CAD build for the part. Positions are in the model's coordinates, mm. A direction names the side the tool comes from. Give positions to 0.01 mm unless a question says otherwise; leave off trailing zeros. Loops run counter-clockwise (first coordinate to the right, second up) from the corner with the lowest first, then second, coordinate; pieces in that order, holes last. Notation, with made-up numbers: (-12, -16.75) - (2, -16.75) arc R14 cw to (2, -1.75) - close; hole circle Ø4 at (21, 28.5). An arc over 180 degrees is marked (long way). Return JSON: item names as keys, results as strings.
from build123d import *

# Parameters (mm, degrees)
SKETCH7_R              = 11
BOSS_EXTRUDE1_DEPTH    = 2.5
SKETCH8_R              = 8.75
SKETCH8_R_2            = 7.6
BOSS_EXTRUDE2_DEPTH    = 1
M14X1_5_TAPPED_HOLE1_D = 12.5
SKETCH13_OUTSIDE_W     = 30.338
SKETCH13_OUTSIDE_H     = 30.338
SKETCH13_OUTSIDE_W_2   = 20
SKETCH13_OUTSIDE_H_2   = 20
CUT_EXTRUDE1_DEPTH     = 17.673332001
M3_TAPPED_HOLE3_REACH  = 24.633
M3_TAPPED_HOLE3_BORE_R = 1.25


with BuildPart() as part:
    # Sketch7 → Boss-Extrude1 (new, symmetric)
    with BuildSketch(Plane.XY):
        Circle(SKETCH7_R)
    extrude(amount=BOSS_EXTRUDE1_DEPTH, both=True)

    # Sketch8 → Boss-Extrude2 (add)
    with BuildSketch(Plane.XY.offset(2.5)):
        Circle(SKETCH8_R)
        Circle(SKETCH8_R_2, mode=Mode.SUBTRACT)
    extrude(amount=BOSS_EXTRUDE2_DEPTH)

    # M14x1.5 Tapped Hole1 (through all)
    with Locations(Plane(origin=(0, 0, -2.5), x_dir=(-1, 0, 0), z_dir=(0, 0, -1))):
        with Locations((0, 0)):
            Hole(M14X1_5_TAPPED_HOLE1_D / 2)

    # Sketch13 outside → Cut-Extrude1 (cut, through all)
    with BuildSketch(Plane(origin=(0, 0, -2.5), x_dir=(-1, 0, 0), z_dir=(0, 0, -1))):
        Rectangle(SKETCH13_OUTSIDE_W, SKETCH13_OUTSIDE_H)
        Rectangle(SKETCH13_OUTSIDE_W_2, SKETCH13_OUTSIDE_H_2, mode=Mode.SUBTRACT)
    extrude(amount=-CUT_EXTRUDE1_DEPTH, mode=Mode.SUBTRACT)

    # M3 Tapped Hole3 bore → M3 Tapped Hole3 (cut, up to next)
    with BuildSketch(Plane(origin=(0, 10, 0), x_dir=(1, 0, 0), z_dir=(0, 1, 0)), mode=Mode.PRIVATE) as m3_tapped_hole3_sk1:
        Circle(M3_TAPPED_HOLE3_BORE_R)
    m3_tapped_hole3_tool1 = extrude(m3_tapped_hole3_sk1.sketch, amount=-M3_TAPPED_HOLE3_REACH, mode=Mode.PRIVATE) & part.part
    add(m3_tapped_hole3_tool1.solids().sort_by_distance((0, 10, 0))[0], mode=Mode.SUBTRACT)


solid = part.part
1. Cut at B-B, the plane z = 2. Write the cut outline in (x, y).
Values follow:
{"outline": "(-10, -4.58) arc R11 ccw to (-4.58, -10) - (4.58, -10) arc R11 ccw to (10, -4.58) - (10, 4.58) arc R11 ccw to (4.58, 10) - (-4.58, 10) arc R11 ccw to (-10, 4.58) - close; hole circle Ø12.5 at (0, 0)"}
2. Which spindle directions (+Z, -Z, +X, -X, +Y, -Y) get a long thin tool onto all of the face, cutting with end or side? Do faces 4 (the face through (7, -6, 2.5)), 5 (the face through (7.817, 7.739, 0.035)), 6 (the face through (-0.27, 8.09, 1.22)). Say none if no direction does.
Values follow:
{"face 4": "+Z", "face 5": "+Z, -Z, +X, +Y", "face 6": "+Y"}
3. Drop flat-ended pins along their axis: P1, Ø2, axis at y = 7.5, z = -1.5, coming from the +X side; P2, Ø5, axis at x = 2.5, y = 2.5, coming from the -Z side. Give the stop position or say it passes through.
Values follow:
{"P1": "stops at x = 8.87", "P2": "passes through"}
4. Cut at C-C, the plane y = 0. Write the cut outline in (x, z), plus the area to 3 significant figures.
Values follow:
{"outline": "(-10, -2.5) - (-6.25, -2.5) - (-6.25, 2.5) - (-7.6, 2.5) - (-7.6, 3.5) - (-8.75, 3.5) - (-8.75, 2.5) - (-10, 2.5) - close; (6.25, -2.5) - (10, -2.5) - (10, 2.5) - (8.75, 2.5) - (8.75, 3.5) - (7.6, 3.5) - (7.6, 2.5) - (6.25, 2.5) - close", "area": "39.8 mm²"}
5. Pull direction X, two halves, no side cores. Call faces 1 (the face through (10, 0, 0)), 2 (the face through (-10, 0, 0)), 3 (the face through (-1.7, -6.2, 2.5)): +X half, -X half, draft (parallel to the pull), parting line (faces both ways), or undercut.
Values follow:
{"face 1": "+X half", "face 2": "-X half", "face 3": "undercut"}
6. Drill centre lines: probe 1 along Y at (x, z) = (0, 2.8); probe 2 along Z at (x, y) = (0, 7.5); probe 3 along Z at (x, y) = (0, 8.7). Where is each one in solid material? Low to high.
Values follow:
{"probe 1": "y = -8.75 to -7.6, 7.6 to 8.75", "probe 2": "z = -2.5 to -1.25, 1.25 to 2.5", "probe 3": "z = -2.5 to -1.25, 1.25 to 3.5"}
7. Cut at A-A, the plane x = 0. Write the cut outline in (y, z).
Values follow:
{"outline": "(-10, -2.5) - (-6.25, -2.5) - (-6.25, 2.5) - (-7.6, 2.5) - (-7.6, 3.5) - (-8.75, 3.5) - (-8.75, 2.5) - (-10, 2.5) - close; (6.25, -2.5) - (10, -2.5) - (10, -1.25) - (6.25, -1.25) - close; (6.25, 1.25) - (10, 1.25) - (10, 2.5) - (8.75, 2.5) - (8.75, 3.5) - (7.6, 3.5) - (7.6, 2.5) - (6.25, 2.5) - close"}
8. Cut at D-D, the plane z = 0. Write the cut outline in (x, y), plus the area to 3 significant figures.
Values follow:
{"outline": "(-10, -4.58) arc R11 ccw to (-4.58, -10) - (4.58, -10) arc R11 ccw to (10, -4.58) - (10, 4.58) arc R11 ccw to (4.58, 10) - (1.25, 10) - (1.25, 6.12) arc R6.25 cw (long way) to (-1.25, 6.12) - (-1.25, 10) - (-4.58, 10) arc R11 ccw to (-10, 4.58) - close", "area": "223 mm²"}
